Print and shaded views of the part. All mm, measured from the part's lowest x, y and z. A direction names the side the tool comes from. Give positions to 0.01 mm unless a question says otherwise; leave off trailing zeros. Loops run counter-clockwise (first coordinate to the right, second up) from the corner with the lowest first, then second, coordinate; pieces in that order, holes last. Notation, with made-up numbers: (-1.75, 23) - (33.25, 23) arc R18 ccw to (33.25, 50) - close; hole circle Ø11 at (-22.75, 50.25). An arc over 180 degrees is marked (long way). Return JSON: item names as keys, results as strings.
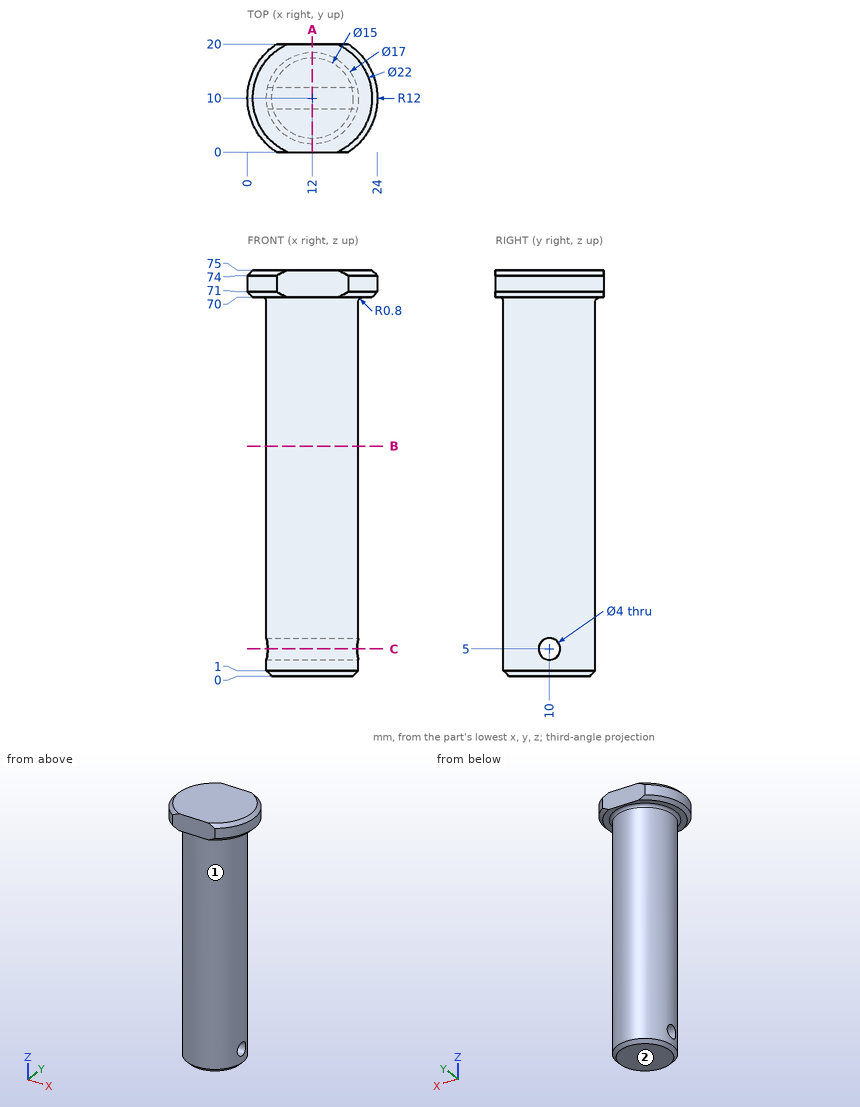
1. Cut at C-C, the plane z = 5. Write the cut outline in (x, y).
Values follow:
{"outline": "(3.74, 8) arc R8.5 ccw to (20.26, 8) - close; (3.74, 12) - (20.26, 12) arc R8.5 ccw to start"}
2. Drop flat-ended pins along their axis: P1, Ø5, axis at x = 19, z = 55.5, coming from the -Y side; P2, Ø1.5, axis at x = 19, z = 37, coming from the -Y side; P3, Ø3, axis at y = 7.5, z = 67, coming from the +X side; P4, Ø3, axis at y = 10, z = 5, coming from the +X side. Give the stop position or say it passes through.
Values follow:
{"P1": "stops at y = 2.79", "P2": "stops at y = 4.24", "P3": "stops at x = 20.44", "P4": "passes through"}
3. Cut at B-B, the plane z = 42.5. Write the cut outline in (x, y), plus the area to 3 significant figures.
Values follow:
{"outline": "circle Ø17 at (12, 10)", "area": "227 mm²"}
4. Which spindle directions (+Z, -Z, +X, -X, +Y, -Y) get a long thin tool onto all of the face, cutting with end or side? Do the marked faces 1 and 2. Say none if no direction does.
Values follow:
{"face 1": "-Z", "face 2": "-Z, +X, -X, +Y, -Y"}
5. Drill centre lines: probe 1 along Y at (x, z) = (11.5, 5); probe 2 along Z at (x, y) = (13.5, 9); probe 3 along Y at (x, z) = (17.25, 5). Where is each one in solid material? Low to high.
Values follow:
{"probe 1": "y = 1.51 to 8, 12 to 18.49", "probe 2": "z = 0 to 3.27, 6.73 to 75", "probe 3": "y = 3.32 to 8, 12 to 16.68"}
6. Cut at A-A, the plane x = 12. Write the cut outline in (y, z), plus the area to 3 significant figures.
Values follow:
{"outline": "(0, 70) - (0.7, 70) arc R0.8 cw to (1.5, 69.2) - (1.5, 1) - (2.5, 0) - (17.5, 0) - (18.5, 1) - (18.5, 69.2) arc R0.8 cw to (19.3, 70) - (20, 70) - (20, 75) - (0, 75) - close; hole circle Ø4 at (10, 5)", "area": "1,280 mm²"}
